from build123d import *

# Parameters (mm, degrees)
U_BRACKET_BODY_DEPTH      = 22
BASE_PLATE_DEPTH          = 10
MOUNTING_HOLES_SKETCH_R   = 4.5
MOUNTING_HOLES_2X_9_DEPTH = 79.102496759


with BuildPart() as part:
    # U-Bracket Profile Sketch → U-Bracket Body (new body)
    with BuildSketch(Plane.XY):
        Polygon((0, 0), (60, 0), (60, 40), (40.761904762, 40), (40.761904762, 32.5), (48.261904762, 32.5), (48.261904762, 20), (13.261904762, 20), (13.261904762, 32.5), (20.761904762, 32.5), (20.761904762, 40), (0, 40), align=None)
    extrude(amount=U_BRACKET_BODY_DEPTH)

    # Base Plate Sketch → Base Plate (add)
    with BuildSketch(Plane.XZ):
        with BuildLine():
            Line((0, 22), (0, 30))
            ThreePointArc((0, 30), (2.928932188, 37.071067812), (10, 40))
            Line((10, 40), (50, 40))
            ThreePointArc((50, 40), (57.071067812, 37.071067812), (60, 30))
            Line((60, 30), (60, 22))
            Line((60, 22), (60, 0))
            Line((60, 0), (0, 0))
            Line((0, 0), (0, 22))
        make_face()
    extrude(amount=-BASE_PLATE_DEPTH)

    # Mounting Holes Sketch → Mounting Holes 2xØ9 (cut, through all)
    with BuildSketch(Plane(origin=(0, 10, 0), x_dir=(1, 0, 0), z_dir=(0, 1, 0))):
        with Locations(Location((10, -30, 0), (0, 0, 270))):
            Circle(MOUNTING_HOLES_SKETCH_R)
        with Locations(Location((50, -30, 0), (0, 0, 270))):
            Circle(MOUNTING_HOLES_SKETCH_R)
    extrude(amount=-MOUNTING_HOLES_2X_9_DEPTH, mode=Mode.SUBTRACT)


solid = part.part
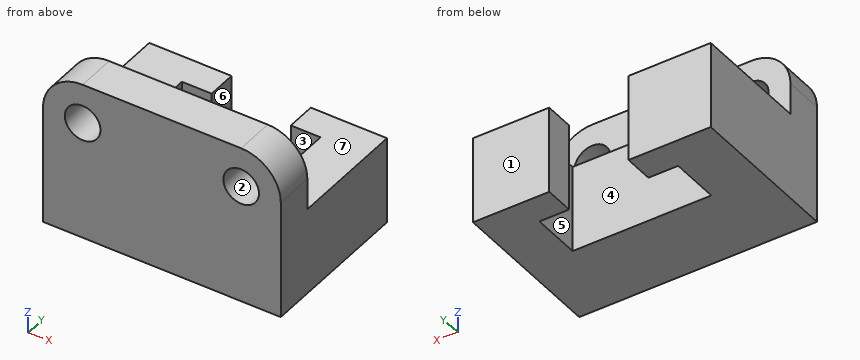
Work out the finished part from the listing and answer in its coordinate system (mm). Face numbers are marked on the shaded views. A direction names the side the tool comes from. Give positions to 0.01 mm unless a question says otherwise; leave off trailing zeros. Write each loop counter-clockwise with the first axis right and the second up, starting at its lowest first coordinate (ties: lowest second). Pieces come first, ordered by that corner, then holes. Notation, with made-up numbers: M -1.75,-8.75 L 26.25,-8.75 A28 ccw 26.25,21.25 Z; hole C 52.25,57.5 d9. An arc over 180 degrees is marked long. Answer as CSV lines item,"result".
Q1. A tool of negligible diameter and unlimited length cuts with its end or side. For the marked faces 5, 6 and 7, from which of +Z, -Z, +X, -X, +Y, -Y can it reach the whole face along a straight path? Write none if from no direction.
A:
face 5,"+Z, -Z"
face 6,"+Z, -Z, +Y"
face 7,"+Z, +X, -X, +Y"
Q2. Given P1, Ø10, axis at x = 25.5, z = 34, coming from the +Y side; P2, Ø6.5, axis at x = 33, z = 9.5, coming from the +Y side; P3, Ø24, axis at x = 31, y = 24, coming from the +Z side, each flat-ended and moving along its own axis, determine where each tip first touches the part or whether it passes through.
A:
P1,"stops at y = 10"
P2,"stops at y = 20"
P3,"stops at z = 22"
Q3. A cutting plane is placed at C-C on z = 14. Write down the section's boundary in (x, y).
A:
outline,"M 0,0 L 60,0 L 60,40 L 40.76,40 L 40.76,32.5 L 48.26,32.5 L 48.26,20 L 13.26,20 L 13.26,32.5 L 20.76,32.5 L 20.76,40 L 0,40 Z"
Q4. The mould has two halves that part along Y. Classify the marked faces 1, 2, 3 and 4: +Y half, -Y half, draft (parallel to the pull), parting line (faces both ways), or undercut.
A:
face 1,"+Y half"
face 2,"draft"
face 3,"undercut"
face 4,"undercut"
Q5. A cutting plane is placed at A-A on y = 35. Write down the section's boundary in (x, z), plus the area to 3 significant figures.
A:
outline,"M 0,0 L 20.76,0 L 20.76,22 L 0,22 Z; M 40.76,0 L 60,0 L 60,22 L 40.76,22 Z"
area,"880 mm²"
Q6. Find the intervals of material crossed by probe 1 along X at (y, z) = (6.75, 30); probe 2 along Y at (x, z) = (42.5, 11.5); probe 3 along X at (y, z) = (38.5, 5), in increasing order. Write a range as [from, to].
A:
probe 1,"x = [0, 5.5], [14.5, 45.5], [54.5, 60]"
probe 2,"y = [0, 20], [32.5, 40]"
probe 3,"x = [0, 20.76], [40.76, 60]"
Q7. A cutting plane is placed at B-B on x = 20. Write down the section's boundary in (y, z).
A:
outline,"M 0,0 L 20,0 L 20,22 L 10,22 L 10,40 L 0,40 Z; M 32.5,0 L 40,0 L 40,22 L 32.5,22 Z"
Q8. A cutting plane is placed at D-D on z = 29. Write down the section's boundary in (x, y).
A:
outline,"M 0,0 L 5.61,0 L 5.61,10 L 0,10 Z; M 14.39,0 L 45.61,0 L 45.61,10 L 14.39,10 Z; M 54.39,0 L 60,0 L 60,10 L 54.39,10 Z"
